from build123d import *

# Parameters (mm, degrees)
BOSS_EXTRUDE1_DEPTH   = 7
M6_TAPPED_HOLE1_D     = 5
M6_TAPPED_HOLE1_DEPTH = 15
M6_TAPPED_HOLE1_TIP   = 1.502151548
M6_TAPPED_HOLE2_D     = 5
M6_TAPPED_HOLE2_DEPTH = 15
M6_TAPPED_HOLE2_TIP   = 1.502151548
CHAMFER1_SIZE         = 1


with BuildPart() as part:
    # Sketch1 → Boss-Extrude1 (new, symmetric)
    with BuildSketch(Plane(origin=(0, 0, 0), x_dir=(0, 0, -1), z_dir=(1, 0, 0))):
        Polygon((0, 0), (0, 25), (-10, 25), (-25, 10), (-25, 0), align=None)
    extrude(amount=BOSS_EXTRUDE1_DEPTH, both=True)

    # M6 Tapped Hole1
    with Locations(Plane(origin=(0, 0, 0), x_dir=(-1, 0, 0), z_dir=(0, -1, 0))):
        with Locations((0, -15)):
            Hole(M6_TAPPED_HOLE1_D / 2, depth=M6_TAPPED_HOLE1_DEPTH)
            with Locations((0, 0, -(M6_TAPPED_HOLE1_DEPTH + M6_TAPPED_HOLE1_TIP / 2))):  # 118° drill point
                Cone(0, M6_TAPPED_HOLE1_D / 2, M6_TAPPED_HOLE1_TIP, mode=Mode.SUBTRACT)

    # M6 Tapped Hole2
    with Locations(Plane(origin=(0, 0, 0), x_dir=(-1, 0, 0), z_dir=(0, 0, -1))):
        with Locations((0, 15)):
            Hole(M6_TAPPED_HOLE2_D / 2, depth=M6_TAPPED_HOLE2_DEPTH)
            with Locations((0, 0, -(M6_TAPPED_HOLE2_DEPTH + M6_TAPPED_HOLE2_TIP / 2))):  # 118° drill point
                Cone(0, M6_TAPPED_HOLE2_D / 2, M6_TAPPED_HOLE2_TIP, mode=Mode.SUBTRACT)

    # Chamfer1
    chamfer1_edges = [part.edges().sort_by_distance(p)[0] for p in [
        (0, 0, 25),
        (0, 25, 0),
        (0, 0, 0),
    ]]
    chamfer(chamfer1_edges, length=CHAMFER1_SIZE)


solid = part.part
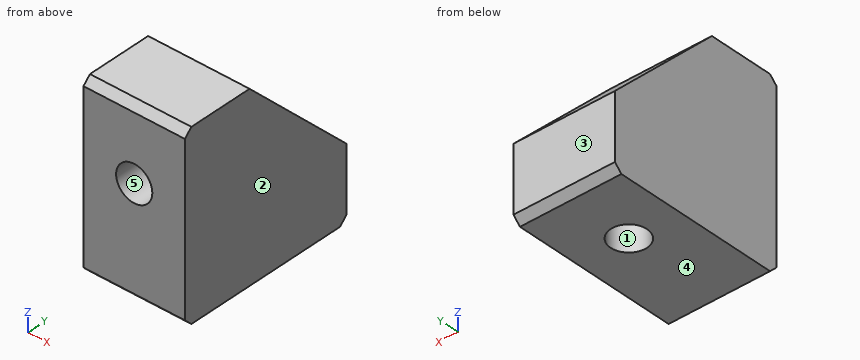
Source: CAD feature listing. Evaluate the final solid. Frame: model axes, mm. Face numbers are marked on the shaded views. A direction names the side the tool comes from. Coordinates: 2 decimals unless noted, no trailing zeros. Order: outer loops, then holes, each group sorted by start corner. A loop starts at its lowest first (then second) coordinate and runs counter-clockwise, first axis right, second up.
Item 1: Cut plane A-A (x = 0). Return loops of the section in (y, z).
Output values:
outline: (0, 1) - (1, 0) - (12.5, 0) - (12.5, 12.5) - (0, 12.5) - close; (0, 17.5) - (15, 17.5) - (15.94, 15.94) - (17.5, 15) - (17.5, 0) - (24, 0) - (25, 1) - (25, 10) - (10, 25) - (1, 25) - (0, 24) - close
Item 2: Cut plane B-B (y = 11.5). Return loops of the section in (x, z), plus the area to 3 significant figures.
Output values:
outline: (-7, 0) - (7, 0) - (7, 23.5) - (-7, 23.5) - close; hole circle Ø5 at (0, 15)
area: 309 mm2
Item 3: Set-up query: the marked faces 1 and 2. Return all of +Z, -Z, +X, -X, +Y, -Y with unobstructed straight access to the full face (end or side cutting, diameter ignored); none if empty.
Output values:
face 1: -Z
face 2: +Z, -Z, +X, +Y, -Y
Item 4: Pull-direction query (Z, two-part tool) for the marked faces 3, 4 and 5; classes: pulls with the +Z half, pulls with the -Z half, needs draft (parallel to the pull), parting line crosses it, or undercut.
Output values:
face 3: needs draft
face 4: pulls with the -Z half
face 5: undercut
Item 5: First-contact query: P1, Ø3, axis at x = 0, y = 15, coming from the -Z side; P2, Ø1, axis at x = 0.5, y = 21, coming from the +Z side. Flat tips, straight axial feed; report the tip coordinate or a pass-through.
Output values:
P1: stops at z = 15.6
P2: stops at z = 14.5
Item 6: Cut plane D-D (x = 5.25). Return loops of the section in (y, z).
Output values:
outline: (0, 1) - (1, 0) - (24, 0) - (25, 1) - (25, 10) - (10, 25) - (1, 25) - (0, 24) - close
Item 7: Material intervals for line 1 (X direction, y = 15, z = 6); line 2 (Y direction, x = 0, z = 3.5), sorted ascending.
Output values:
line 1: x = -7 to -2.5, 2.5 to 7
line 2: y = 0 to 12.5, 17.5 to 25
